```python
from build123d import *

# Parameters (mm, degrees)
SKETCH1_R          = 5
BOSS_EXTRUDE_DEPTH = 9.5
SKETCH2_OUTSIDE_W  = 308.252
SKETCH2_OUTSIDE_H  = 305.896
SKETCH2_OUTSIDE_R  = 7.616693426
CUT_EXTRUDE1_DEPTH = 38
CUT_EXTRUDE1_DRAFT = -75
SKETCH3_OUTSIDE_W  = 308.252
SKETCH3_OUTSIDE_H  = 305.896
SKETCH3_OUTSIDE_R  = 7.616693426
CUT_EXTRUDE2_DEPTH = 38
CUT_EXTRUDE2_DRAFT = -75
CHAMFER1_SIZE      = 0.2


with BuildPart() as part:
    # Sketch1 → Boss-Extrude (new body)
    with BuildSketch(Plane.XY):
        Polygon((4.3975, 7.616693426), (-4.3975, 7.616693426), (-8.795, 0), (-4.3975, -7.616693426), (4.3975, -7.616693426), (8.795, 0), align=None)
        Circle(SKETCH1_R, mode=Mode.SUBTRACT)
    extrude(amount=BOSS_EXTRUDE_DEPTH)


with BuildPart() as cut_extrude1_tool:
    # Sketch2 outside → Cut-Extrude1 (with draft: the straight prism first)
    with BuildSketch(Plane(origin=(0, 0, 0), x_dir=(-1, 0, 0), z_dir=(0, 0, -1))):
        Rectangle(SKETCH2_OUTSIDE_W, SKETCH2_OUTSIDE_H)
        Circle(SKETCH2_OUTSIDE_R, mode=Mode.SUBTRACT)
    extrude(amount=-CUT_EXTRUDE1_DEPTH)
    # Cut-Extrude1: the draft: its side faces are tilted about the plane it starts from
    cut_extrude1_sides = [cut_extrude1_tool.faces().sort_by_distance(p)[0] for p in [
        (0, -152.948, 19),
        (-154.126, 0, 19),
        (0, 152.948, 19),
        (154.126, 0, 19),
        (7.616693426, 0, 19),
    ]]
    draft(cut_extrude1_sides, Plane(origin=(0, 0, 0), x_dir=(-1, 0, 0), z_dir=(0, 0, -1)), CUT_EXTRUDE1_DRAFT)


with BuildPart() as part_1:
    add(part.part)

    # Cut-Extrude1: cut by cut_extrude1_tool
    add(cut_extrude1_tool.part, mode=Mode.SUBTRACT)


with BuildPart() as cut_extrude2_tool:
    # Sketch3 outside → Cut-Extrude2 (with draft: the straight prism first)
    with BuildSketch(Plane.XY.offset(9.5)):
        Rectangle(SKETCH3_OUTSIDE_W, SKETCH3_OUTSIDE_H)
        Circle(SKETCH3_OUTSIDE_R, mode=Mode.SUBTRACT)
    extrude(amount=-CUT_EXTRUDE2_DEPTH)
    # Cut-Extrude2: the draft: its side faces are tilted about the plane it starts from
    cut_extrude2_sides = [cut_extrude2_tool.faces().sort_by_distance(p)[0] for p in [
        (0, -152.948, -9.5),
        (154.126, 0, -9.5),
        (0, 152.948, -9.5),
        (-154.126, 0, -9.5),
        (-7.616693426, 0, -9.5),
    ]]
    draft(cut_extrude2_sides, Plane.XY.offset(9.5), CUT_EXTRUDE2_DRAFT)


with BuildPart() as part_2:
    add(part_1.part)

    # Cut-Extrude2: cut by cut_extrude2_tool
    add(cut_extrude2_tool.part, mode=Mode.SUBTRACT)

    # Chamfer1
    chamfer1_edges = [part_2.edges().sort_by_distance(p)[0] for p in [
        (-5, 0, 0),
        (-5, 0, 9.5),
    ]]
    chamfer(chamfer1_edges, length=CHAMFER1_SIZE)


solid = part_2.part
```
The model under review builds one solid part; all positions refer to its coordinate system, in mm. Round coordinates to 2 decimals unless told otherwise and drop trailing zeros. Loops run counter-clockwise (first coordinate to the right, second up) from the corner with the lowest first, then second, coordinate; pieces in that order, holes last. Notation, with made-up numbers: (13.5, -38.75) -> (58.5, -38.75) arc R23 ccw to (58.5, -1.75) -> close; hole circle Ø6 at (88.25, -13). An arc over 180 degrees is marked (long way). Answer as a JSON object with one key per item and string values. Group by question number.
1) For pin 1 Ø2 at (y, z) = (-2, 4.5) entering from +X, flat-tipped, find the tip position at first contact; note if it passes through.
2) Mouldability with a two-part tool opening along X and no side actions: class faces 1 (the face through (-3.966, -6.83, 9.425)), 2 (the face through (-1.08, -4.88, 4.69)), 3 (the face through (7.898, -0.019, 9.425)) as released by +X, released by -X, zero draft, split by the parting line, or undercut.
3) For line 1 (Y direction, x = 0, z = 2.75); line 2 (X direction, y = 4, z = 3.5); line 3 (X direction, y = 6.5, z = 7.25), list the stretches that pass through material, from the lowest coordinate up. Write a range as [from, to].
4) We need section A-A on z = 4.75. Write out the cut boundary in (x, y) (1 decimal).
Result set:
{
 "1": {"pin 1": "x = 8.22"},
 "2": {"face 1": "released by -X", "face 2": "undercut", "face 3": "released by +X"},
 "3": {"line 1": "[-7.62, -5], [5, 7.62]", "line 2": "[-6.49, -3], [3, 6.49]", "line 3": "[-5.04, 5.04]"},
 "4": {"outline": "(-8.8, 0) -> (-4.4, -7.6) -> (4.4, -7.6) -> (8.8, 0) -> (4.4, 7.6) -> (-4.4, 7.6) -> close; hole circle Ø10 at (0, 0)"}
}
